The listing builds one solid part. Answer for the finished solid, in the listing's coordinates (mm). Give positions to 0.01 mm unless a question says otherwise; leave off trailing zeros. Write each loop counter-clockwise with the first axis right and the second up, starting at its lowest first coordinate (ties: lowest second). Pieces come first, ordered by that corner, then holes. Notation, with made-up numbers: (-21, 14) - (-5, 14) arc R7 ccw to (-5, 18) - close; hole circle Ø2 at (35.25, -10). An arc over 180 degrees is marked (long way). Return JSON: item names as keys, results as strings.
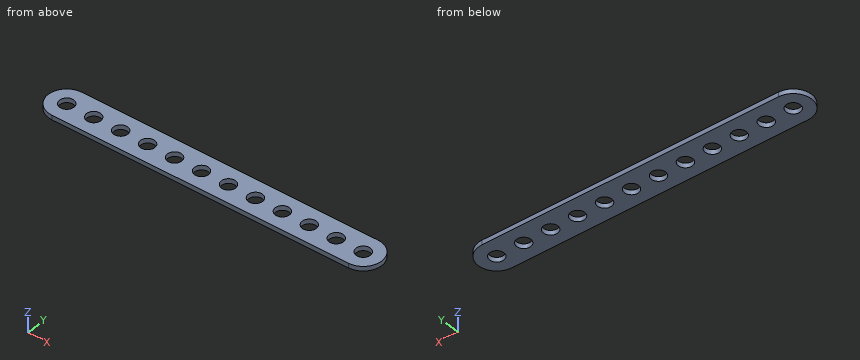
from build123d import *

# Parameters (mm, degrees)
SKETCH_1_R      = 1.55
EXTRUDE_1_DEPTH = 1


with BuildPart() as part:
    # 草图1 → 凸台-拉伸1 (new body)
    with BuildSketch(Plane.XY):
        with BuildLine():
            Line((0, 4), (64, 4))
            ThreePointArc((64, 4), (68, 0), (64, -4))
            Line((64, -4), (0, -4))
            ThreePointArc((0, -4), (-4, 0), (0, 4))
        make_face()
        Circle(SKETCH_1_R, mode=Mode.SUBTRACT)
        with Locations((5.818181818, 0)):
            Circle(SKETCH_1_R, mode=Mode.SUBTRACT)
        with Locations((11.636363636, 0)):
            Circle(SKETCH_1_R, mode=Mode.SUBTRACT)
        with Locations((17.454545455, 0)):
            Circle(SKETCH_1_R, mode=Mode.SUBTRACT)
        with Locations((23.272727273, 0)):
            Circle(SKETCH_1_R, mode=Mode.SUBTRACT)
        with Locations((29.090909091, 0)):
            Circle(SKETCH_1_R, mode=Mode.SUBTRACT)
        with Locations((34.909090909, 0)):
            Circle(SKETCH_1_R, mode=Mode.SUBTRACT)
        with Locations((40.727272727, 0)):
            Circle(SKETCH_1_R, mode=Mode.SUBTRACT)
        with Locations((46.545454545, 0)):
            Circle(SKETCH_1_R, mode=Mode.SUBTRACT)
        with Locations((52.363636364, 0)):
            Circle(SKETCH_1_R, mode=Mode.SUBTRACT)
        with Locations((58.181818182, 0)):
            Circle(SKETCH_1_R, mode=Mode.SUBTRACT)
        with Locations((64, 0)):
            Circle(SKETCH_1_R, mode=Mode.SUBTRACT)
    extrude(amount=EXTRUDE_1_DEPTH)


solid = part.part
Item 1: Consider L1, parallel to Y at x = 0, z = 0.5; L2, parallel to Y at x = 22.5, z = 0.4; L3, parallel to X at y = 3.25, z = 0.4. Determine where each line is inside the solid, lowest interval first.
Answer below:
{"L1": "y = -4 to -1.55, 1.55 to 4", "L2": "y = -4 to -1.34, 1.34 to 4", "L3": "x = -2.33 to 66.33"}
Item 2: A cutting plane is placed at B-B on z = 0.85. Give the number of separate pieces and of enclosed holes in the cut face, then the cut area to 3 significant figures.
Answer below:
{"separate pieces": "1", "enclosed holes": "12", "area": "472 mm²"}
Item 3: A cutting plane is placed at A-A on x = 6. Determine the outline of the cut face in (y, z), then the cut area to 3 significant figures.
Answer below:
{"outline": "(-4, 0) - (-1.54, 0) - (-1.54, 1) - (-4, 1) - close; (1.54, 0) - (4, 0) - (4, 1) - (1.54, 1) - close", "area": "4.92 mm²"}
Item 4: A cutting plane is placed at D-D on x = 34. Determine the outline of the cut face in (y, z), then the cut area to 3 significant figures.
Answer below:
{"outline": "(-4, 0) - (-1.26, 0) - (-1.26, 1) - (-4, 1) - close; (1.26, 0) - (4, 0) - (4, 1) - (1.26, 1) - close", "area": "5.49 mm²"}
